```python
from build123d import *

# Parameters (mm, degrees)
BOSS_EXTRUDE1_DEPTH    = 10
BOSS_EXTRUDE2_DEPTH    = 10
M16X1_5_TAPPED_HOLE1_D = 14.5


with BuildPart() as part:
    # Sketch1 → Boss-Extrude1 (new body)
    with BuildSketch(Plane(origin=(0, 0, 0), x_dir=(1, 0, 0), z_dir=(0, 1, 0))):
        Polygon((8.660254038, -15), (17.320508076, 0), (8.660254038, 15), (-8.660254038, 15), (-17.320508076, 0), (-8.660254038, -15), align=None)
    extrude(amount=BOSS_EXTRUDE1_DEPTH)

    # Sketch4 → Revolve1 (revolve)
    with BuildSketch(Plane.XY, mode=Mode.PRIVATE) as revolve1_sk:
        Polygon((0, 0), (17.320508076, 0), (35, -103), (0, -103), align=None)
    revolve(revolve1_sk.sketch.rotate(Axis((0, -103, 0), (0, 1, 0)), 90), axis=Axis((0, -103, 0), (0, 1, 0)))

    # Sketch7 → Boss-Extrude2 (add)
    with BuildSketch(Plane.XZ.offset(103)):
        Polygon((17.5, 30.310889132), (-17.5, 30.310889132), (-35, 0), (-17.5, -30.310889132), (17.5, -30.310889132), (35, 0), align=None)
    extrude(amount=BOSS_EXTRUDE2_DEPTH)

    # M16x1.5 Tapped Hole1 (through all)
    with Locations(Plane(origin=(0, 10, 0), x_dir=(1, 0, 0), z_dir=(0, 1, 0))):
        with Locations((0, 0)):
            Hole(M16X1_5_TAPPED_HOLE1_D / 2)


solid = part.part
```
Geometry: final body of the model. Coordinates: model frame, mm. A direction names the side the tool comes from. Round coordinates to 2 decimals unless told otherwise and drop trailing zeros. Order: outer loops, then holes, each group sorted by start corner. A loop starts at its lowest first (then second) coordinate and runs counter-clockwise, first axis right, second up. Notation, with made-up numbers: (50.5, 8) -> (100.5, 8) arc R5 ccw to (100.5, 16) -> close; hole circle Ø3 at (54.5, 63.5). An arc over 180 degrees is marked (long way). Use CSV: the item, a comma, the result in double quotes. Start each with the question number.
1) Section B-B (x = 0). Return the cut outline in (y, z), and give its area (3 significant figures).
2) Section A-A (y = -105). Return the cut outline in (x, z), and give its area (3 significant figures).
3) Set-up query: faces 1 (the face through (26.372, -107.93, 14.943)), 2 (the face through (-28, -103, 16)), 3 (the face through (-13.05, 4.93, 7.4)). Return all of +Z, -Z, +X, -X, +Y, -Y with unobstructed straight access to the full face (end or side cutting, diameter ignored); none if empty.
4) Material intervals for line 1 along Z through (x, y) = (-2.5, -14.5); line 2 along Y through (x, z) = (13.5, -9.5); line 3 along X through (y, z) = (-35.5, 3.5), sorted ascending. Write a range as from..to.
5) First-contact query: pin 1 Ø5 at (x, y) = (3.5, 7) entering from -Z; pin 2 Ø4 at (x, y) = (17.5, -36.5) entering from -Z; pin 3 Ø2.5 at (x, z) = (0, 32.5) entering from -Y. Flat tips, straight axial feed; report the tip coordinate or a pass-through.
6) Section C-C (y = -22). Return the cut outline in (x, z), and give its area (3 significant figures).
7) Section D-D (y = -68.5). Return the cut outline in (x, z).
8) Draft query along X for faces 4 (the face through (0, 5, -15)), 5 (the face through (-26.372, -107.93, -14.943)), 6 (the face through (-3.35, -52.36, 6.43)), 7 (the face through (26.128, -107.93, -15.368)). Return one class per face: +X half, -X half, draft (parallel to the pull), parting line (faces both ways), or undercut.
Returned:
1,outline,"(-113, -30.31) -> (-103, -30.31) -> (-103, -35) -> (0, -17.32) -> (0, -15) -> (10, -15) -> (10, -7.25) -> (-113, -7.25) -> close; (-113, 7.25) -> (10, 7.25) -> (10, 15) -> (0, 15) -> (0, 17.32) -> (-103, 35) -> (-103, 30.31) -> (-113, 30.31) -> close"
1,area,"4,510 mm²"
2,outline,"(-35, 0) -> (-17.5, -30.31) -> (17.5, -30.31) -> (35, 0) -> (17.5, 30.31) -> (-17.5, 30.31) -> close; hole circle Ø14.5 at (0, 0)"
2,area,"3,020 mm²"
3,face 1,"+Z, +X, -Y"
3,face 2,"+Z, -X, -Y"
3,face 3,"+Z, -X, +Y"
4,line 1,"z = -19.65..-6.81, 6.81..19.65"
4,line 2,"y = -113..0"
4,line 3,"x = -23.15..-6.35, 6.35..23.15"
5,pin 1,"stops at z = -15"
5,pin 2,"stops at z = -17.84"
5,pin 3,"stops at y = -103"
6,outline,"circle Ø42.19 at (0, 0); hole circle Ø14.5 at (0, 0)"
6,area,"1,230 mm²"
7,outline,"circle Ø58.16 at (0, 0); hole circle Ø14.5 at (0, 0)"
8,face 4,"draft"
8,face 5,"-X half"
8,face 6,"undercut"
8,face 7,"+X half"
